Check sheet for the modelled part. Datum: model origin and axes. Units: mm. Face numbers are marked on the shaded views. A direction names the side the tool comes from. Give positions to 0.01 mm unless a question says otherwise; leave off trailing zeros. Loops run counter-clockwise (first coordinate to the right, second up) from the corner with the lowest first, then second, coordinate; pieces in that order, holes last. Notation, with made-up numbers: M 61.25,7.25 L 69.25,7.25 A18 cw 69.25,32.25 Z; hole C 17.5,3 d1. An arc over 180 degrees is marked long. Write each question's results on one line, items separated by ' | '. Start each with the question number.
1. Tool access check on the marked faces 1 and 2. Record the directions out of +Z, -Z, +X, -X, +Y, -Y that give a thin tool (end or side, any length) a straight path to the whole face; none if there is none.
2. Material ranges on line 1 along Z through (x, y) = (15, -0.25); line 2 along X through (y, z) = (3.5, 0.25); line 3 along Y through (x, z) = (18, 2.75), recorded low to high.
3. Go/stop test with flat-tipped pins: pin 1 (1 mm diameter, centred on y = -3.5, z = -1.5, fed in from -X); pin 2 (1 mm diameter, centred on x = 16.5, z = -1, fed in from -Y). Record where each tip stops, or that it passes through.
4. Sectioned sample at A-A on x = 27.5. Record the cut outline in (y, z), and give its area (3 significant figures).
```python
from build123d import *

# Parameters (mm, degrees)
BASEHEAD_DEPTH = 4
SKETCH5_R      = 3
BASEBODY_DEPTH = 45
CHAMFER1_SIZE  = 0.3


with BuildPart() as part:
    # Sketch2 → BaseHead (new body)
    with BuildSketch(Plane(origin=(0, 0, 0), x_dir=(0, 0, -1), z_dir=(1, 0, 0))):
        Polygon((0, -5.773502692), (5, -2.886751346), (5, 2.886751346), (0, 5.773502692), (-5, 2.886751346), (-5, -2.886751346), align=None)
    extrude(amount=BASEHEAD_DEPTH)

    # Sketch3 → BearingFace (revolve, cut)
    with BuildSketch(Plane.XY, mode=Mode.PRIVATE) as bearingface_sk:
        Polygon((4, 5.773502692), (4, 4.37), (3.5, 4.87), (3.5, 5.773502692), align=None)
    revolve(bearingface_sk.sketch.rotate(Axis((-0.957090588, 0, 0), (1, 0, 0)), 90), axis=Axis((-0.957090588, 0, 0), (1, 0, 0)), mode=Mode.SUBTRACT)

    # Sketch4 → HeadChamfer (revolve, cut)
    with BuildSketch(Plane.XY):
        Polygon((0, 5.773502692), (0.281531956, 5.773502692), (0, 5), align=None)
    revolve(axis=Axis((-0.493528746, 0, 0), (1, 0, 0)), mode=Mode.SUBTRACT)

    # Sketch5 → BaseBody (add)
    with BuildSketch(Plane(origin=(4, 0, 0), x_dir=(0, 0, -1), z_dir=(1, 0, 0))):
        with Locations(Location((0, 0, 0), (0, 0, 180))):
            Circle(SKETCH5_R)
    extrude(amount=BASEBODY_DEPTH)

    # Chamfer1
    chamfer1_edges = [part.edges().sort_by_distance(p)[0] for p in [
        (49, 0, -3),
    ]]
    chamfer(chamfer1_edges, length=CHAMFER1_SIZE)


solid = part.part
```
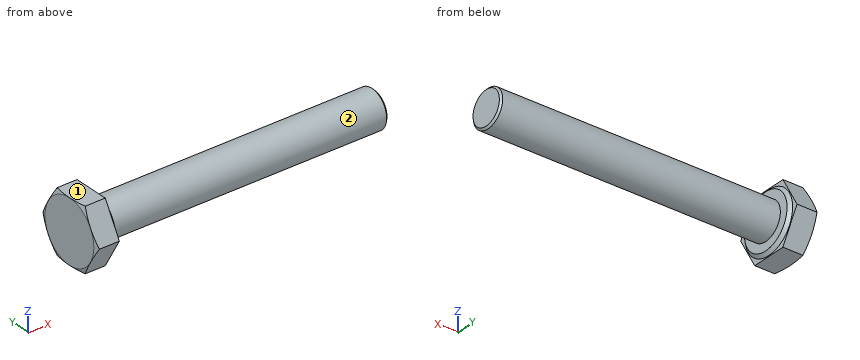
Output values:
1) face 1: +Z, +X, -X, +Y, -Y | face 2: +X
2) line 1: -2.99 to 2.99 | line 2: 0 to 4 | line 3: -1.2 to 1.2
3) pin 1: x = 0 | pin 2: y = -2.96
4) outline: C 0,0 d6 | area: 28.3 mm2
